Can you work these out from the model? Positions are in its coordinate system, mm. Coordinates: 2 decimals unless noted, no trailing zeros. Order: outer loops, then holes, each group sorted by start corner. A loop starts at its lowest first (then second) coordinate and runs counter-clockwise, first axis right, second up. Notation, with made-up numbers: (89, 59.5) -> (97, 59.5) arc R11 ccw to (97, 71.5) -> close; hole circle Ø3 at (73, 25.25). An arc over 180 degrees is marked (long way). Answer as CSV lines item,"result".
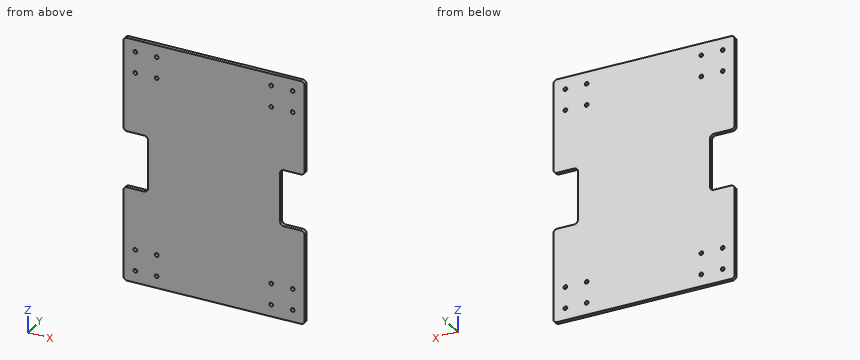
from build123d import *

# Parameters (mm, degrees)
SKETCH1_W           = 480
SKETCH1_H           = 650
BOSS_EXTRUDE1_DEPTH = 10
SKETCH3_W           = 130
SKETCH3_H           = 150
CUT_EXTRUDE1_DEPTH  = 10
FILLET1_R           = 10
FILLET3_R           = 10
SKETCH5_R           = 5
CUT_EXTRUDE2_DEPTH  = 10


with BuildPart() as part:
    # Sketch1 → Boss-Extrude1 (new body)
    with BuildSketch(Plane(origin=(0, 0, 0), x_dir=(1, 0, 0), z_dir=(0, 1, 0))):
        Rectangle(SKETCH1_W, SKETCH1_H)
    extrude(amount=BOSS_EXTRUDE1_DEPTH)

    # Sketch3 → Cut-Extrude1 (cut)
    with BuildSketch(Plane(origin=(0, 10, 0), x_dir=(1, 0, 0), z_dir=(0, 1, 0))):
        with Locations((240, 0)):
            Rectangle(SKETCH3_W, SKETCH3_H)
        with Locations((-240, 0)):
            Rectangle(SKETCH3_W, SKETCH3_H)
    extrude(amount=-CUT_EXTRUDE1_DEPTH, mode=Mode.SUBTRACT)

    # Fillet1
    fillet1_edges = [part.edges().sort_by_distance(p)[0] for p in [
        (240, 5, -75),
        (175, 5, -75),
        (240, 5, 75),
        (175, 5, 75),
        (-240, 5, 75),
        (-175, 5, 75),
        (-175, 5, -75),
        (-240, 5, -75),
    ]]
    fillet(fillet1_edges, radius=FILLET1_R)

    # Fillet3
    fillet3_edges = [part.edges().sort_by_distance(p)[0] for p in [
        (240, 5, 325),
        (-240, 5, 325),
        (-240, 5, -325),
        (240, 5, -325),
    ]]
    fillet(fillet3_edges, radius=FILLET3_R)

    # Sketch5 → Cut-Extrude2 (cut)
    with BuildSketch(Plane(origin=(0, 10, 0), x_dir=(1, 0, 0), z_dir=(0, 1, 0))):
        with Locations(Location((-208.284271247, -293.284271247, 0), (0, 0, 270))):
            Circle(SKETCH5_R)
        with Locations(Location((-208.284271247, -236.715728753, 0), (0, 0, 270))):
            Circle(SKETCH5_R)
        with Locations(Location((-151.715728753, -236.715728753, 0), (0, 0, 270))):
            Circle(SKETCH5_R)
        with Locations(Location((-151.715728753, -293.284271247, 0), (0, 0, 270))):
            Circle(SKETCH5_R)
        with Locations(Location((208.284271247, -293.284271247, 0), (0, 0, 270))):
            Circle(SKETCH5_R)
        with Locations(Location((151.715728753, -293.284271247, 0), (0, 0, 270))):
            Circle(SKETCH5_R)
        with Locations(Location((151.715728753, -236.715728753, 0), (0, 0, 270))):
            Circle(SKETCH5_R)
        with Locations(Location((208.284271247, -236.715728753, 0), (0, 0, 270))):
            Circle(SKETCH5_R)
        with Locations(Location((-208.284271247, 236.715728753, 0), (0, 0, 270))):
            Circle(SKETCH5_R)
        with Locations(Location((208.284271247, 293.284271247, 0), (0, 0, 270))):
            Circle(SKETCH5_R)
        with Locations(Location((208.284271247, 236.715728753, 0), (0, 0, 270))):
            Circle(SKETCH5_R)
        with Locations(Location((151.715728753, 293.284271247, 0), (0, 0, 270))):
            Circle(SKETCH5_R)
        with Locations(Location((151.715728753, 236.715728753, 0), (0, 0, 270))):
            Circle(SKETCH5_R)
        with Locations(Location((-151.715728753, 293.284271247, 0), (0, 0, 270))):
            Circle(SKETCH5_R)
        with Locations(Location((-208.284271247, 293.284271247, 0), (0, 0, 270))):
            Circle(SKETCH5_R)
        with Locations(Location((-151.715728753, 236.715728753, 0), (0, 0, 270))):
            Circle(SKETCH5_R)
    extrude(amount=-CUT_EXTRUDE2_DEPTH, mode=Mode.SUBTRACT)


solid = part.part
Q1. Imagine slicing it at B-B (y = 4.5). Give the number of separate pieces and of enclosed holes in the cut face, and give its area (3 significant figures).
Solution:
separate pieces,"1"
enclosed holes,"16"
area,"291,000 mm2"
Q2. For P1, Ø9, axis at x = 208.28, z = -293.28, coming from the -Y side; P2, Ø2, axis at y = 8, z = 65.5, coming from the -X side; P3, Ø3, axis at y = 3.5, z = -9.5, coming from the -X side, each with a flat end and sliding along its axis, tell me the tip position at first contact or that it passes through.
Solution:
P1,"through"
P2,"x = -175.11"
P3,"x = -175"
Q3. If I drill on line 1 (Z direction, x = 209, y = 7.5); line 2 (Z direction, x = -190.5, y = 8); line 3 (X direction, y = 4.75, z = 20), over which ranges is the centre line in solid material (lowest first)?
Solution:
line 1,"-325 to -298.23, -288.34 to -241.66, -231.77 to -75, 75 to 231.77, 241.66 to 288.34, 298.23 to 325"
line 2,"-325 to -75, 75 to 325"
line 3,"-175 to 175"
Q4. Imagine slicing it at A-A (z = 1.5). List the corners of the cut face in (x, y) for me, and give its area (3 significant figures).
Solution:
outline,"(-175, 0) -> (175, 0) -> (175, 10) -> (-175, 10) -> close"
area,"3,500 mm2"
